Part model, mm, in its own coordinate system. Face numbers are marked on the shaded views. A direction names the side the tool comes from. Round coordinates to 2 decimals unless told otherwise and drop trailing zeros. Write each loop counter-clockwise with the first axis right and the second up, starting at its lowest first coordinate (ties: lowest second). Pieces come first, ordered by that corner, then holes. Notation, with made-up numbers: M 83,83.5 L 117,83.5 A23 cw 117,109.5 Z; hole C 14,75.5 d2. An arc over 180 degrees is marked long. Answer as a JSON object with one key per item and string values. Group by question number.
1. Which spindle directions (+Z, -Z, +X, -X, +Y, -Y) get a long thin tool onto all of the face, cutting with end or side? Do the marked faces 1, 2, 3 and 4. Say none if no direction does.
2. Band-saw the part on D-D, the plane y = -9. Write the cut outline in (x, z), plus the area to 3 significant figures.
3. Two-plate mould, pull along Y, no slides. Class the marked faces 5, 6 and 7: +Y half, -Y half, draft (parallel to the pull), parting line (faces both ways), or undercut.
4. Drill centre lines: line 1 (Y direction, x = 0, z = 9.5); line 2 (X direction, y = -4, z = 0.75); line 3 (Z direction, x = 12.5, y = -19.5). Where is each one in solid material? Low to high. Write a range as from..to.
5. Band-saw the part on A-A, the plane x = 0. Write the cut outline in (y, z).
6. Band-saw the part on C-C, the plane z = 3. Count the separate pieces of the cut face and the enclosed holes in it, plus the area to 3 significant figures.
7. Drop flat-ended pins along their axis: pin 1 (6.5 mm diameter, centred on x = -8.66, y = -5, fed in from +Z); pin 2 (4 mm diameter, centred on y = 6.5, z = 12.5, fed in from -X); pin 3 (3 mm diameter, centred on y = 12, z = 5, fed in from +X). Give the stop position or say it passes through.
8. Band-saw the part on B-B, the plane y = -19. Write the cut outline in (x, z).
from build123d import *

# Parameters (mm, degrees)
SLOTTED_FLANGE_48_DEPTH = 4
HUB_SKETCH_R            = 14
HUB_28_DEPTH            = 7
HUB_HOLES_SKETCH_R      = 2
HUB_HOLES_6X_4_DEPTH    = 30
SPIGOT_SKETCH_R         = 4
SPIGOT_8_DEPTH          = 5
BORE_SKETCH_R           = 3
BORE_6_DEPTH            = 50
FLANGE_HOLES_SKETCH_R   = 1.5
FLANGE_HOLES_3X_3_DEPTH = 30


with BuildPart() as part:
    # Flange Profile Sketch → Slotted Flange Ø48 (new body)
    with BuildSketch(Plane.XY):
        with BuildLine():
            Line((4.846767643, -23.505506661), (2.865571245, -17.112023963))
            ThreePointArc((2.865571245, -17.112023963), (0, -15), (-2.865571245, -17.112023963))
            Line((-2.865571245, -17.112023963), (-4.846767643, -23.505506661))
            ThreePointArc((-4.846767643, -23.505506661), (-20.784609691, -12), (-22.779749719, 7.555329425))
            Line((-22.779749719, 7.555329425), (-16.252233084, 6.074354487))
            ThreePointArc((-16.252233084, 6.074354487), (-12.990381057, 7.5), (-13.38666184, 11.037669476))
            Line((-13.38666184, 11.037669476), (-17.932982076, 15.950177236))
            ThreePointArc((-17.932982076, 15.950177236), (0, 24), (17.932982076, 15.950177236))
            Line((17.932982076, 15.950177236), (13.38666184, 11.037669476))
            ThreePointArc((13.38666184, 11.037669476), (12.990381057, 7.5), (16.252233084, 6.074354487))
            Line((16.252233084, 6.074354487), (22.779749719, 7.555329425))
            ThreePointArc((22.779749719, 7.555329425), (20.784609691, -12), (4.846767643, -23.505506661))
        make_face()
    extrude(amount=SLOTTED_FLANGE_48_DEPTH)

    # Hub Sketch → Hub Ø28 (add)
    with BuildSketch(Plane.XY.offset(4)):
        Circle(HUB_SKETCH_R)
    extrude(amount=HUB_28_DEPTH)

    # Hub Holes Sketch → Hub Holes 6xØ4 (cut)
    with BuildSketch(Plane.XY.offset(11)):
        with Locations((0, 10)):
            Circle(HUB_HOLES_SKETCH_R)
        with Locations((8.660254038, 5)):
            Circle(HUB_HOLES_SKETCH_R)
        with Locations((8.660254038, -5)):
            Circle(HUB_HOLES_SKETCH_R)
        with Locations((0, -10)):
            Circle(HUB_HOLES_SKETCH_R)
        with Locations((-8.660254038, -5)):
            Circle(HUB_HOLES_SKETCH_R)
        with Locations((-8.660254038, 5)):
            Circle(HUB_HOLES_SKETCH_R)
    extrude(amount=-HUB_HOLES_6X_4_DEPTH, mode=Mode.SUBTRACT)

    # Spigot Sketch → Spigot Ø8 (add)
    with BuildSketch(Plane.XY.offset(11)):
        Circle(SPIGOT_SKETCH_R)
    extrude(amount=SPIGOT_8_DEPTH)

    # Bore Sketch → Bore Ø6 (cut)
    with BuildSketch(Plane.XY.offset(16)):
        Circle(BORE_SKETCH_R)
    extrude(amount=-BORE_6_DEPTH, mode=Mode.SUBTRACT)

    # Flange Holes Sketch → Flange Holes 3xØ3 (cut)
    with BuildSketch(Plane.XY.offset(4)):
        with Locations((15.588457268, -9)):
            Circle(FLANGE_HOLES_SKETCH_R)
        with Locations((0, 18)):
            Circle(FLANGE_HOLES_SKETCH_R)
        with Locations((-15.588457268, -9)):
            Circle(FLANGE_HOLES_SKETCH_R)
    extrude(amount=-FLANGE_HOLES_3X_3_DEPTH, mode=Mode.SUBTRACT)


solid = part.part
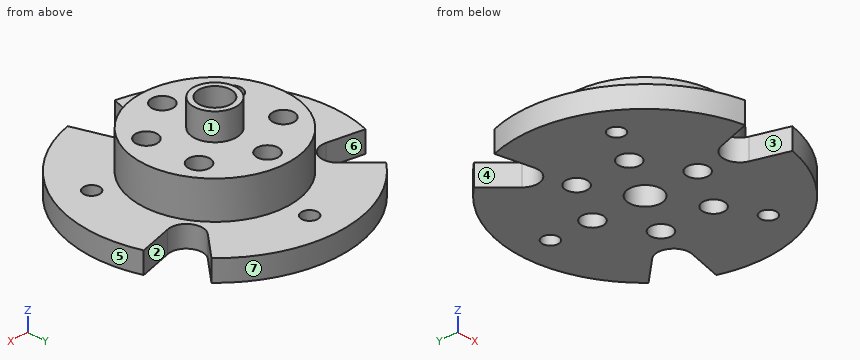
Worked answers:
{
 "1": {"face 1": "+Z", "face 2": "+Z, -Z", "face 3": "+Z, -Z, -Y", "face 4": "+Z, -Z, -X"},
 "2": {"outline": "M -22.25,0 L -17.09,0 L -17.09,4 L -22.25,4 Z; M -14.09,0 L -1.73,0 L -1.73,11 L -10.72,11 L -10.72,4 L -14.09,4 Z; M 1.73,0 L 14.09,0 L 14.09,4 L 10.72,4 L 10.72,11 L 1.73,11 Z; M 17.09,0 L 22.25,0 L 22.25,4 L 17.09,4 Z", "area": "266 mm^2"},
 "3": {"face 5": "parting line", "face 6": "undercut", "face 7": "+Y half"},
 "4": {"line 1": "y = -14..-12, -8..-3, 3..8, 12..14", "line 2": "x = -23.66..-10.39, -6.93..6.93, 10.39..23.66", "line 3": "z = 0..4"},
 "5": {"outline": "M -15,0 L -12,0 L -12,11 L -14,11 L -14,4 L -15,4 Z; M -8,0 L -3,0 L -3,16 L -4,16 L -4,11 L -8,11 Z; M 3,0 L 8,0 L 8,11 L 4,11 L 4,16 L 3,16 Z; M 12,0 L 16.5,0 L 16.5,4 L 14,4 L 14,11 L 12,11 Z; M 19.5,0 L 24,0 L 24,4 L 19.5,4 Z"},
 "6": {"separate pieces": "1", "enclosed holes": "10", "area": "1,500 mm^2"},
 "7": {"pin 1": "stops at z = 11", "pin 2": "stops at x = -13.01", "pin 3": "stops at x = 15.31"},
 "8": {"outline": "M -14.66,0 L -3.45,0 L -3.45,4 L -14.66,4 Z; M 3.45,0 L 14.66,0 L 14.66,4 L 3.45,4 Z"}
}
